Could you check a few things on this model? Use its own coordinates, in mm. A direction names the side the tool comes from. Give positions to 0.01 mm unless a question says otherwise; leave off trailing zeros. Order: outer loops, then holes, each group sorted by start corner. A loop starts at its lowest first (then second) coordinate and runs counter-clockwise, first axis right, second up.
(1) Imagine slicing it at D-D, the plane z = 37.5. Write out the boundary of the cut face in (x, y).
(2) If I drill on probe 1 along Y at (x, z) = (-27.5, 22.5); probe 2 along Y at (x, z) = (132, 21.5); probe 3 along X at (y, z) = (48, 21), over which ranges is the centre line in solid material (lowest first)?
(3) Imagine slicing it at A-A, the plane z = 8. Write out the boundary of the cut face in (x, y), then the cut area to 3 significant figures.
(4) Will these pins go through, and if not, where does the flat tip stop? pin 1 (15 mm diameter, centred on y = 68, z = 13, fed in from +X); pin 2 (6 mm diameter, centred on y = 47, z = 17.5, fed in from -X); pin 3 (2 mm diameter, centred on x = -51, z = 19.5, fed in from +Y).
(5) On a 3-axis mill with a long thin cutter (end or side, diameter ignored), from which of +Z, -Z, +X, -X, +Y, -Y can I reach the whole of each face in a straight line? I mean faces 1 (the flat face through (68, -49, 50)), 2 (the flat face through (-150.5, 66, 12)), 3 (the flat face through (-11.62, -19.74, 37.33)). Say none if no direction works.
(6) Imagine slicing it at B-B, the plane x = 81.5. Write out the boundary of the cut face in (y, z).
(7) Imagine slicing it at C-C, the plane y = -60.5. Write out the boundary of the cut face in (x, z).
from build123d import *

# Parameters (mm, degrees)
EXTRUDE_1_DEPTH     = 50
SKETCH_2_W          = 128.455604429
SKETCH_2_H          = 25
SKETCH_2_W_2        = 42.23428711
CUT_EXTRUDE_1_DEPTH = 49


with BuildPart() as part:
    # 草图1 → 凸台-拉伸1 (new body)
    with BuildSketch(Plane.XY):
        with BuildLine():
            Line((-158.499845276, 75.499845276), (-158.499845276, 56.452935893))
            ThreePointArc((-158.499845276, 56.452935893), (-151.653526546, 34.694072336), (-133.581521944, 20.77563589))
            Line((-133.581521944, 20.77563589), (146.746117531, -82.011165251))
            Line((146.746117531, -82.011165251), (149.500154724, -83.020978889))
            Line((149.500154724, -83.020978889), (149.500154724, -74.500154724))
            Line((149.500154724, -74.500154724), (-130.827484751, 28.286646417))
            ThreePointArc((-130.827484751, 28.286646417), (-145.094856805, 39.274885717), (-150.499845276, 56.452935893))
            Line((-150.499845276, 56.452935893), (-150.499845276, 75.499845276))
            Line((-150.499845276, 75.499845276), (-158.499845276, 75.499845276))
        make_face()
    extrude(amount=EXTRUDE_1_DEPTH)

    # 草图2 → 切除-拉伸1 (cut)
    with BuildSketch(Plane(origin=(-9.115968963, -24.861733537, 0), x_dir=(0.9388763158866098, -0.3442546491584201, 0), z_dir=(-0.3442546491584201, -0.9388763158866098, 0))):
        with Locations((-68.340834223, 37.5)):
            Rectangle(SKETCH_2_W, SKETCH_2_H)
        with Locations((-153.685779993, 37.5)):
            Rectangle(SKETCH_2_W_2, SKETCH_2_H)
    extrude(amount=-CUT_EXTRUDE_1_DEPTH, mode=Mode.SUBTRACT)


solid = part.part
Answer block:
1. outline: (-12.98, -23.45) - (149.5, -83.02) - (149.5, -74.5) - (-10.22, -15.93) - close
2. probe 1: y = -18.12 to -9.6
2. probe 2: y = -76.6 to -68.08
2. probe 3: x = -157.55 to -149.28
3. outline: (-158.5, 56.45) arc R38 ccw to (-133.58, 20.78) - (149.5, -83.02) - (149.5, -74.5) - (-130.83, 28.29) arc R30 cw to (-150.5, 56.45) - (-150.5, 75.5) - (-158.5, 75.5) - close
3. area: 2,880 mm2
4. pin 1: stops at x = -150.5
4. pin 2: stops at x = -157.95
4. pin 3: stops at y = -0.62
5. face 1: +Z, +X, -X, +Y, -Y
5. face 2: +Z, -Z, +X, +Y
5. face 3: +Z, -X, +Y
6. outline: (-58.09, 0) - (-49.57, 0) - (-49.57, 50) - (-58.09, 50) - close
7. outline: (88.08, 0) - (111.32, 0) - (111.32, 50) - (88.08, 50) - close
